```python
from build123d import *

# Parameters (mm, degrees)
BOSS_EXTRUDE1_DEPTH = 1100
CUT_EXTRUDE1_DEPTH  = 1295.604186615
SKETCH3_W           = 20
SKETCH3_H           = 560
BOSS_EXTRUDE2_DEPTH = 60
SKETCH4_R           = 11
CUT_EXTRUDE2_DEPTH  = 1288.953803519


with BuildPart() as part:
    # Sketch1 → Boss-Extrude1 (new body)
    with BuildSketch(Plane.XY):
        Polygon((360, 0), (-360, 0), (-360, 20), (-335, 20), (-335, 580), (-315, 580), (-315, 20), (315, 20), (315, 580), (335, 580), (335, 20), (360, 20), align=None)
    extrude(amount=BOSS_EXTRUDE1_DEPTH)

    # Sketch2 → Cut-Extrude1 (cut, through all)
    with BuildSketch(Plane(origin=(0, 0, 0), x_dir=(-1, 0, 0), z_dir=(0, 0, -1))):
        Polygon((-360, 20), (-59.240800915, 20), (-59.240800915, 755.063041929), (647.427412598, 706.251760561), (560.651801276, -150.657401245), (-360, -188.621731198), (-684.035873625, -70.661134557), align=None)
    extrude(amount=-CUT_EXTRUDE1_DEPTH, mode=Mode.SUBTRACT)

    # Sketch3 → Boss-Extrude2 (add)
    with BuildSketch(Plane(origin=(335, 0, 0), x_dir=(0, 0, -1), z_dir=(1, 0, 0))):
        with Locations((-1090, 300)):
            Rectangle(SKETCH3_W, SKETCH3_H)
    extrude(amount=BOSS_EXTRUDE2_DEPTH)

    # Sketch4 → Cut-Extrude2 (cut, through all)
    with BuildSketch(Plane(origin=(0, 0, 1080), x_dir=(-1, 0, 0), z_dir=(0, 0, -1))):
        with Locations((-365, 450)):
            Circle(SKETCH4_R)
        with Locations((-365, 150)):
            Circle(SKETCH4_R)
    extrude(amount=-CUT_EXTRUDE2_DEPTH, mode=Mode.SUBTRACT)


solid = part.part
```
Could you check a few things on this model? Use its own coordinates, in mm. A direction names the side the tool comes from. Round coordinates to 2 decimals unless told otherwise and drop trailing zeros. Loops run counter-clockwise (first coordinate to the right, second up) from the corner with the lowest first, then second, coordinate; pieces in that order, holes last. Notation, with made-up numbers: (-16, 54.25) - (35, 54.25) arc R22 cw to (35, 79.25) - close; hole circle Ø5 at (51.5, -39). An arc over 180 degrees is marked (long way). Answer as CSV lines item,"result".
1. I want a section at B-B on x = 365. List the corners of the cut face in (y, z) for me.
Filled in:
outline,"(20, 1080) - (139, 1080) - (139, 1100) - (20, 1100) - close; (161, 1080) - (439, 1080) - (439, 1100) - (161, 1100) - close; (461, 1080) - (580, 1080) - (580, 1100) - (461, 1100) - close"
2. For pin 1 Ø10 at (y, z) = (394, 974.5) entering from +X; pin 2 Ø13 at (x, y) = (365, 450) entering from -Z; pin 3 Ø1.5 at (x, y) = (383.5, 93.5) entering from -Z, each with a flat end and sliding along its axis, tell me the tip position at first contact or that it passes through.
Filled in:
pin 1,"stops at x = 335"
pin 2,"passes through"
pin 3,"stops at z = 1080"
3. I want a section at A-A on y = 150. List the corners of the cut face in (x, z) for me.
Filled in:
outline,"(315, 0) - (335, 0) - (335, 1080) - (354, 1080) - (354, 1100) - (315, 1100) - close; (376, 1080) - (395, 1080) - (395, 1100) - (376, 1100) - close"
4. I want a section at C-C on z = 87. List the corners of the cut face in (x, y) for me.
Filled in:
outline,"(315, 20) - (335, 20) - (335, 580) - (315, 580) - close"
5. On a 3-axis mill with a long thin cutter (end or side, diameter ignored), from which of +Z, -Z, +X, -X, +Y, -Y can I reach the whole of each face in a straight line? I mean faces 5 (the face through (331, 580, 593)), 6 (the face through (335, 304, 532)). Say none if no direction works.
Filled in:
face 5,"+Z, -Z, +X, -X, +Y"
face 6,"-Z, +X, +Y, -Y"
6. We'd pull the mould along X, two halves only. Please class faces 1 (the face through (331, 20, 593)), 2 (the face through (373.73, 443.31, 1089.86)), 3 (the face through (315, 296, 542)), 4 (the face through (376, 150, 1090)): +X half, -X half, draft (parallel to the pull), parting line (faces both ways), or undercut.
Filled in:
face 1,"draft"
face 2,"undercut"
face 3,"-X half"
face 4,"undercut"
7. Please list where these lines run through material, in increasing order: line 1 along Y through (x, z) = (365, 1084); line 2 along Z through (x, y) = (373, 113.5); line 3 along X through (y, z) = (160, 1054). Write a range as [from, to].
Filled in:
line 1,"y = [20, 139], [161, 439], [461, 580]"
line 2,"z = [1080, 1100]"
line 3,"x = [315, 335]"
